Build history of the part. All positions in model axes, mm. A direction names the side the tool comes from. Give positions to 0.01 mm unless a question says otherwise; leave off trailing zeros. Order: outer loops, then holes, each group sorted by start corner. A loop starts at its lowest first (then second) coordinate and runs counter-clockwise, first axis right, second up. Notation, with made-up numbers: M -17,-36.75 L -10,-36.75 A34 ccw -10,-4.75 Z; hole C 53.5,82.5 d3. An arc over 180 degrees is marked long. One line per item, written item: value. Start each with the question number.
from build123d import *

# Parameters (mm, degrees)
BASE_PLATE_DEPTH              = 12
SUPPORT_WEB_DEPTH             = 12
WEB_GUSSET_RIB_REACH          = 205.838
WEB_GUSSET_RIB_SKETCH_WALL_W  = 462.836477652
WEB_GUSSET_RIB_SKETCH_WALL_H  = 12
SIDE_GUSSET_RIB_REACH         = 205.838
SIDE_GUSSET_RIB_SKETCH_WALL_W = 483.925921336
SIDE_GUSSET_RIB_SKETCH_WALL_H = 12
GREASE_BOSS_16_REACH          = 209.425
GREASE_BOSS_16_END_RADIUS     = 41
GREASE_BOSS_SKETCH_R          = 8
LUBE_HOLE_SKETCH_R            = 2
LUBE_HOLE_DEPTH               = 35
GREASE_BOSS_CHAMFER_4X45_SIZE = 4


with BuildPart() as part:
    # Base Plate Sketch → Base Plate (new body)
    with BuildSketch(Plane(origin=(0, 0, 0), x_dir=(1, 0, 0), z_dir=(0, 1, 0))):
        with BuildLine():
            Line((-90, -35), (-90, -8))
            Line((-90, -8), (-78, -8))
            ThreePointArc((-78, -8), (-70, 0), (-78, 8))
            Line((-78, 8), (-90, 8))
            Line((-90, 8), (-90, 35))
            Line((-90, 35), (-26, 70))
            Line((-26, 70), (0, 70))
            Line((0, 70), (125, 35))
            Line((125, 35), (125, 8))
            Line((125, 8), (113, 8))
            ThreePointArc((113, 8), (105, 0), (113, -8))
            Line((113, -8), (125, -8))
            Line((125, -8), (125, -35))
            Line((125, -35), (0, -70))
            Line((0, -70), (-26, -70))
            Line((-26, -70), (-90, -35))
        make_face()
    extrude(amount=BASE_PLATE_DEPTH)



with BuildPart() as body_2:
    # Bearing Boss Profile → Bearing Boss (revolve)
    with BuildSketch(Plane.XY, mode=Mode.PRIVATE) as bearing_boss_sk:
        Polygon((53, 104), (-32, 104), (-32, 63), (3, 63), (3, 79), (53, 79), align=None)
    revolve(bearing_boss_sk.sketch.rotate(Axis((53, 104, 0), (-1, 0, 0)), 180), axis=Axis((53, 104, 0), (-1, 0, 0)))

    # Stepped Bore Profile → Stepped Bore (revolve, cut)
    with BuildSketch(Plane.XY, mode=Mode.PRIVATE) as stepped_bore_sk:
        Polygon((-32, 128), (3, 128), (3, 124), (53, 124), (53, 104), (-32, 104), align=None)
    revolve(stepped_bore_sk.sketch.rotate(Axis((-32, 104, 0), (1, 0, 0)), 90), axis=Axis((-32, 104, 0), (1, 0, 0)), mode=Mode.SUBTRACT)


with BuildPart() as part_1:
    add(part.part)

    add(body_2.part)  # Support Web merges body 2
    # Support Web Sketch → Support Web (add)
    with BuildSketch(Plane(origin=(0, 0, 0), x_dir=(0, 0, -1), z_dir=(1, 0, 0))):
        with BuildLine():
            Line((-70, 12), (-41, 104))
            ThreePointArc((-41, 104), (0, 63), (41, 104))
            Line((41, 104), (70, 12))
            Line((70, 12), (35, 12))
            Line((35, 12), (8, 12))
            Line((8, 12), (-8, 12))
            Line((-8, 12), (-35, 12))
            Line((-35, 12), (-70, 12))
        make_face()
    extrude(amount=-SUPPORT_WEB_DEPTH)

    # Web Gusset Rib Sketch wall → Web Gusset Rib (add, up to next)
    with BuildSketch(Plane(origin=(-39.5, 37.5, 0), x_dir=(-0.282166323992, -0.959365501571, 0), z_dir=(0.959365501571, -0.282166323992, 0)), mode=Mode.PRIVATE) as web_gusset_rib_sk1:
        Rectangle(WEB_GUSSET_RIB_SKETCH_WALL_W, WEB_GUSSET_RIB_SKETCH_WALL_H)
    web_gusset_rib_tool1 = extrude(web_gusset_rib_sk1.sketch, amount=WEB_GUSSET_RIB_REACH, mode=Mode.PRIVATE) - part_1.part
    add(web_gusset_rib_tool1.solids().sort_by_distance((-39.5, 37.5, 0))[0])

    # Side Gusset Rib Sketch wall → Side Gusset Rib (add, up to next)
    with BuildSketch(Plane(origin=(69, 45.5, 0), x_dir=(0.430978873925, -0.90236201728, 0), z_dir=(0.90236201728, 0.430978873925, 0)), mode=Mode.PRIVATE) as side_gusset_rib_sk1:
        Rectangle(SIDE_GUSSET_RIB_SKETCH_WALL_W, SIDE_GUSSET_RIB_SKETCH_WALL_H)
    side_gusset_rib_tool1 = extrude(side_gusset_rib_sk1.sketch, amount=-SIDE_GUSSET_RIB_REACH, mode=Mode.PRIVATE) - part_1.part
    add(side_gusset_rib_tool1.solids().sort_by_distance((69, 45.5, 0))[0])

    # Grease Boss Ø16: up to this cylinder (the profile starts outside it)
    grease_boss_16_end = Plane(origin=(-14.5, 104, 0), z_dir=(1, 0, 0)) * Cylinder(GREASE_BOSS_16_END_RADIUS, 501.85, mode=Mode.PRIVATE)
    # Grease Boss Sketch → Grease Boss Ø16 (add, up to the surface)
    with BuildSketch(Plane(origin=(0, 150, 0), x_dir=(1, 0, 0), z_dir=(0, 1, 0)), mode=Mode.PRIVATE) as grease_boss_16_sk1:
        with Locations(Location((-14.5, 0, 0), (0, 0, 270))):
            Circle(GREASE_BOSS_SKETCH_R)
    grease_boss_16_tool1 = extrude(grease_boss_16_sk1.sketch, amount=-GREASE_BOSS_16_REACH, mode=Mode.PRIVATE) - grease_boss_16_end
    add(grease_boss_16_tool1.solids().sort_by_distance((-14.5, 150, 0))[0])

    # Lube Hole Sketch → Lube Hole (cut)
    with BuildSketch(Plane(origin=(0, 150, 0), x_dir=(1, 0, 0), z_dir=(0, 1, 0))):
        with Locations(Location((-14.5, 0, 0), (0, 0, 270))):
            Circle(LUBE_HOLE_SKETCH_R)
    extrude(amount=-LUBE_HOLE_DEPTH, mode=Mode.SUBTRACT)

    # Grease Boss Chamfer 4x45°
    grease_boss_chamfer_4x45_edges = [part_1.edges().sort_by_distance(p)[0] for p in [
        (-14.5, 150, -2),
    ]]
    chamfer(grease_boss_chamfer_4x45_edges, length=GREASE_BOSS_CHAMFER_4X45_SIZE)


solid = part_1.part
1) Pull direction Z, two halves, no side cores. Call faces 1 (the flat face through (-5.92, 58.64, -55.3)), 2 (the flat face through (0, 48, -38)), 3 (the flat face through (-84, 6, 8)): pulls with the +Z half, pulls with the -Z half, needs draft (parallel to the pull), parting line crosses it, or undercut.
2) Slice it at B-B (x = 36.5). List the corners of the cut face in (y, z), plus the area to 3 significant figures.
3) Slice it at D-D (z = -45.5). List the corners of the cut face in (x, y), plus the area to 3 significant figures.
4) Slice it at A-A (y = 88.5). List the corners of the cut face in (x, z).
5) Drill centre lines: line 1 (Z direction, x = -14.5, y = 104); line 2 (Z direction, x = 28.5, y = 104); line 3 (Y direction, x = -23, z = 0). Where is each one in solid material? Low to high.
6) Drop flat-ended pins along their axis: P1, Ø19, axis at y = 52.5, z = 29.5, coming from the -X side; P2, Ø1, axis at x = 50, y = 23.5, coming from the -Z side; P3, Ø3.5, axis at x = 120.5, y = 4.5, coming from the +Z side. Give the stop position or say it passes through.
7) Tool access for faces 4 (the flat face through (3, 122, 18)), 5 (the flat face through (37, 44, 6)), 6 (the flat face through (53, 93, -17)), 7 (the flat face through (-26, 37, -6)): list every direction of +Z, -Z, +X, -X, +Y, -Y with a clear straight run to the whole face (end or side of a thin tool).
8) Slice it at C-C (z = -14). List the corners of the cut face in (x, y).
Results list:
1. face 1: pulls with the -Z half
1. face 2: needs draft
1. face 3: undercut
2. outline: M 0,-59.78 L 12,-59.78 L 12,-6 L 79.73,-6 A25 ccw long 79.73,6 L 12,6 L 12,59.78 L 0,59.78 Z; hole C 104,0 d40
2. area: 2,950 mm²
3. outline: M -70.8,0 L 87.5,0 L 87.5,12 L 0,12 L 0,89.72 L -12,89.72 L -12,12 L -70.8,12 Z
3. area: 2,830 mm²
4. outline: M -32,-37.96 L -12,-37.96 L -12,-45.89 L 0,-45.89 L 0,-37.96 L 3,-37.96 L 3,-19.62 L 53,-19.62 L 53,-12.64 L 3,-12.64 L 3,-18.32 L -32,-18.32 Z; M -32,18.32 L 3,18.32 L 3,12.64 L 53,12.64 L 53,19.62 L 3,19.62 L 3,37.96 L 0,37.96 L 0,45.89 L -12,45.89 L -12,37.96 L -32,37.96 Z
5. line 1: z = -41 to -24, 24 to 41
5. line 2: z = -25 to -20, 20 to 25
5. line 3: y = 0 to 80, 128 to 145
6. P1: stops at x = -12
6. P2: stops at z = -6
6. P3: stops at z = 36.75
7. face 4: +X
7. face 5: +Z, +X
7. face 6: +Z, -Z, +X, +Y
7. face 7: -Z, -X
8. outline: M -90,0 L 125,0 L 125,12 L 0,12 L 0,65.46 L 3,65.46 L 3,83.29 L 53,83.29 L 53,89.72 L 3,89.72 L 3,84.51 L -32,84.51 L -32,65.46 L -12,65.46 L -12,12 L -90,12 Z; M -32,123.49 L 3,123.49 L 3,118.28 L 53,118.28 L 53,124.71 L 3,124.71 L 3,142.54 L -32,142.54 Z
